Geometry check sheet. Reference: the model listing, model coordinates, mm. Face numbers are marked on the shaded views. Give positions to 0.01 mm unless a question says otherwise; leave off trailing zeros. Write each loop counter-clockwise with the first axis right and the second up, starting at its lowest first coordinate (ties: lowest second). Pieces come first, ordered by that corner, then holes. Notation, with made-up numbers: (81, -1) -> (98, -1) arc R16 cw to (98, 12) -> close; hole circle Ø6 at (11.25, -30). An arc over 180 degrees is marked (long way). Write item = value, one per line. Start each with the question number.
1. Cross-section at B-B, the plane x = 0. Record the cut outline in (y, z).
2. Cross-section at A-A, the plane z = 0. Record the cut outline in (x, y), plus the area to 3 significant figures.
3. Cross-section at C-C, the plane y = 3.5. Record the cut outline in (x, z).
4. Depth check by flat-ended pin: P1, Ø6, axis at x = -2.5, y = 7.5, coming from the -Z side; P2, Ø5, axis at x = -33, y = 7, coming from the -Z side. Enter the tip coordinate at first touch or a pass-through.
5. Thickness scan on line 1 along X through (y, z) = (4.25, 0); line 2 along X through (y, z) = (6.25, -22); line 3 along Z through (x, y) = (-10, 1). Record the ranges inside material, lowest first.
6. Mould release check, pull along Z, two halves, no side actions. Record for the marked faces 1, 2 and 3: pulls with the +Z half, pulls with the -Z half, needs draft (parallel to the pull), parting line crosses it, or undercut.
```python
from build123d import *

# Parameters (mm, degrees)
SKETCH_1_R      = 50
SKETCH_1_R_2    = 40
EXTRUDE_1_DEPTH = 10
FILLET_1_R      = 1


with BuildPart() as part:
    # 草图1 → 凸台-拉伸1 (new body)
    with BuildSketch(Plane(origin=(0, 0, 0), x_dir=(1, 0, 0), z_dir=(0, 1, 0))):
        with Locations(Location((0, 0, 0), (0, 0, 270))):
            Circle(SKETCH_1_R)
        with Locations(Location((0, 0, 0), (0, 0, 270))):
            Circle(SKETCH_1_R_2, mode=Mode.SUBTRACT)
    extrude(amount=EXTRUDE_1_DEPTH)

    # 圆角1
    fillet_1_edges = [part.edges().sort_by_distance(p)[0] for p in [
        (0, 0, -50),
        (0, 10, -50),
        (0, 0, -40),
        (0, 10, -40),
    ]]
    fillet(fillet_1_edges, radius=FILLET_1_R)


solid = part.part
```
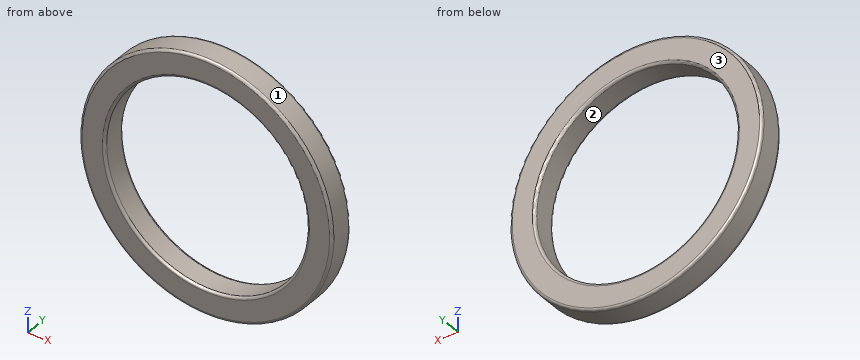
Answers:
q1.outline = (0, -49) arc R1 ccw to (1, -50) -> (9, -50) arc R1 ccw to (10, -49) -> (10, -41) arc R1 ccw to (9, -40) -> (1, -40) arc R1 ccw to (0, -41) -> close; (0, 41) arc R1 ccw to (1, 40) -> (9, 40) arc R1 ccw to (10, 41) -> (10, 49) arc R1 ccw to (9, 50) -> (1, 50) arc R1 ccw to (0, 49) -> close
q2.outline = (-50, 1) arc R1 ccw to (-49, 0) -> (-41, 0) arc R1 ccw to (-40, 1) -> (-40, 9) arc R1 ccw to (-41, 10) -> (-49, 10) arc R1 ccw to (-50, 9) -> close; (40, 1) arc R1 ccw to (41, 0) -> (49, 0) arc R1 ccw to (50, 1) -> (50, 9) arc R1 ccw to (49, 10) -> (41, 10) arc R1 ccw to (40, 9) -> close
q2.area = 198 mm^2
q3.outline = circle Ø100 at (0, 0); hole circle Ø80 at (0, 0)
q4.P1 = -50
q4.P2 = -39.62
q5.line_1 = -50 to -40, 40 to 50
q5.line_2 = -44.9 to -33.41, 33.41 to 44.9
q5.line_3 = -48.99 to -38.73, 38.73 to 48.99
q6.face_1 = parting line crosses it
q6.face_2 = undercut
q6.face_3 = needs draft
